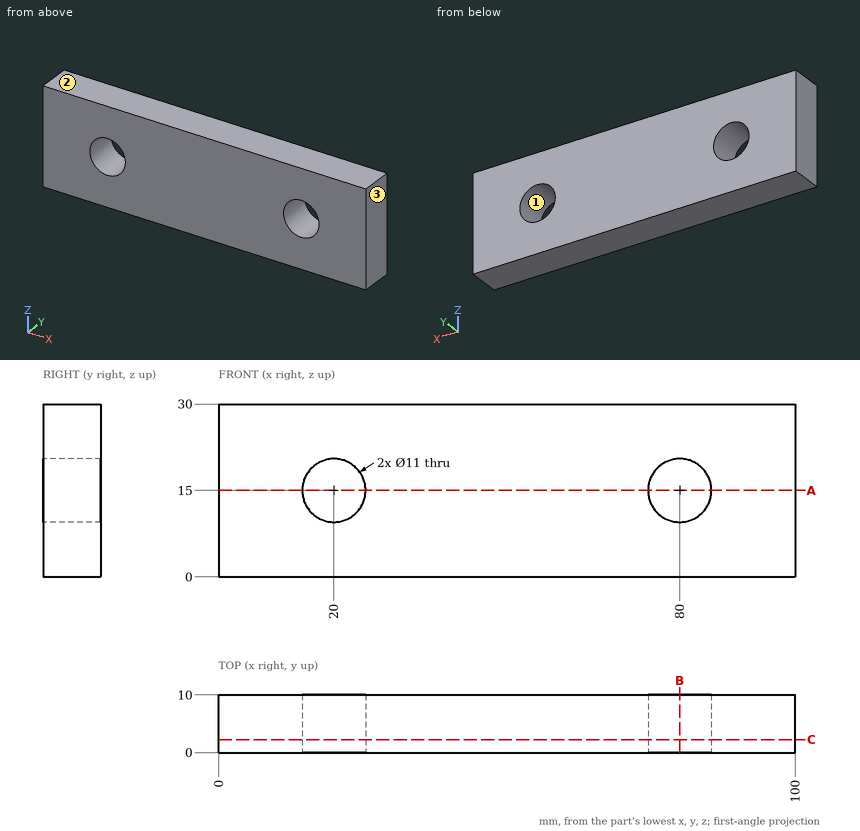
Input: dimensioned drawing with shaded views. Units: mm. Origin: part minimum x, y, z. Coordinates: 2 decimals unless noted, no trailing zeros. Loops run counter-clockwise (first coordinate to the right, second up) from the corner with the lowest first, then second, coordinate; pieces in that order, holes last. Notation, with made-up numbers: (89.25, -38) -> (110.25, -38) arc R7 cw to (110.25, -25) -> close; hole circle Ø9 at (60.25, 88.5). An arc over 180 degrees is marked (long way). Use a Markdown table: item, result. Add a question column.
(1) Section query A-A, the plane z = 15. Return loops of the section in (x, y), plus the area to 3 significant figures.
(2) Line query: line 1 along Z through (x, y) = (20, 7.25); line 2 along X through (y, z) = (8.5, 19); line 3 along X through (y, z) = (2, 17.5). Output: solid intervals per line, ascending.
(3) Mould query, pull axis Z, two halves, no side actions, for the marked faces 1, 2 and 3. Classes: pulls with the +Z half, pulls with the -Z half, needs draft (parallel to the pull), parting line crosses it, or undercut.
(4) Section query B-B, the plane x = 80. Return loops of the section in (y, z).
(5) Section query C-C, the plane y = 2.25. Return loops of the section in (x, z), plus the area to 3 significant figures.
Answer:
| question | item | result |
|---|---|---|
| 1 | outline | (0, 0) -> (14.5, 0) -> (14.5, 10) -> (0, 10) -> close; (25.5, 0) -> (74.5, 0) -> (74.5, 10) -> (25.5, 10) -> close; (85.5, 0) -> (100, 0) -> (100, 10) -> (85.5, 10) -> close |
| 1 | area | 780 mm^2 |
| 2 | line 1 | z = 0 to 9.5, 20.5 to 30 |
| 2 | line 2 | x = 0 to 16.23, 23.77 to 76.23, 83.77 to 100 |
| 2 | line 3 | x = 0 to 15.1, 24.9 to 75.1, 84.9 to 100 |
| 3 | face 1 | undercut |
| 3 | face 2 | pulls with the +Z half |
| 3 | face 3 | needs draft |
| 4 | outline | (0, 0) -> (10, 0) -> (10, 9.5) -> (0, 9.5) -> close; (0, 20.5) -> (10, 20.5) -> (10, 30) -> (0, 30) -> close |
| 5 | outline | (0, 0) -> (100, 0) -> (100, 30) -> (0, 30) -> close; hole circle Ø11 at (20, 15); hole circle Ø11 at (80, 15) |
| 5 | area | 2,810 mm^2 |
